from build123d import *

# Parameters (mm, degrees)
WEB_RECESS_SKETCH_R       = 100
WEB_RECESS_200_DEPTH      = 28
LIGHTENING_HOLES_SKETCH_R = 18
LIGHTENING_HOLES_4X_DEPTH = 11
HUB_SKETCH_R              = 25
HUB_50_DEPTH              = 35
BORE_SKETCH_R             = 12.5
BORE_25_DEPTH             = 35
KEYWAY_SKETCH_W           = 3
KEYWAY_SKETCH_H           = 6
KEYWAY_6X3_DEPTH          = 35


with BuildPart() as part:
    # Pulley Profile Sketch → Pulley Body 3-Groove (revolve)
    with BuildSketch(Plane.XY, mode=Mode.PRIVATE) as pulley_body_3_groove_sk:
        Polygon((-38.155633051, 12.5), (38.155633051, 12.5), (38.155633051, 125), (33.155633051, 125), (26.604168834, 107), (20.629224678, 107.05281598), (14.096983906, 125), (9.096983906, 125), (2.5, 106.874935681), (-2.5, 106.874935681), (-9.096983906, 125), (-14.096983906, 125), (-20.629224678, 107.05281598), (-26.604168834, 107), (-33.155633051, 125), (-38.155633051, 125), align=None)
    revolve(pulley_body_3_groove_sk.sketch.rotate(Axis((-177.514342584, 0, 0), (1, 0, 0)), 90), axis=Axis((-177.514342584, 0, 0), (1, 0, 0)))

    # Web Recess Sketch → Web Recess Ø200 (cut)
    with BuildSketch(Plane(origin=(38.155633051, 0, 0), x_dir=(0, 0, -1), z_dir=(1, 0, 0))):
        Circle(WEB_RECESS_SKETCH_R)
    web_recess_200 = extrude(amount=-WEB_RECESS_200_DEPTH, mode=Mode.SUBTRACT)

    # Web Recess Mirror: Web Recess Ø200 across plane
    add(web_recess_200.mirror(Plane(origin=(0, 0, 0), x_dir=(0, 0, 1), z_dir=(1, 0, 0))), mode=Mode.SUBTRACT)

    # Lightening Holes Sketch → Lightening Holes 4x (cut, symmetric)
    with BuildSketch(Plane(origin=(0, 0, 0), x_dir=(0, 0, -1), z_dir=(1, 0, 0))):
        with Locations((0, 62.5)):
            Circle(LIGHTENING_HOLES_SKETCH_R)
        with Locations((62.5, 0)):
            Circle(LIGHTENING_HOLES_SKETCH_R)
        with Locations((0, -62.5)):
            Circle(LIGHTENING_HOLES_SKETCH_R)
        with Locations((-62.5, 0)):
            Circle(LIGHTENING_HOLES_SKETCH_R)
    extrude(amount=LIGHTENING_HOLES_4X_DEPTH, both=True, mode=Mode.SUBTRACT)

    # Hub Sketch → Hub Ø50 (add, symmetric)
    with BuildSketch(Plane(origin=(0, 0, 0), x_dir=(0, 0, -1), z_dir=(1, 0, 0))):
        with Locations(Location((0, 0, 0), (0, 0, 180))):
            Circle(HUB_SKETCH_R)
    extrude(amount=HUB_50_DEPTH, both=True)

    # Bore Sketch → Bore Ø25 (cut, symmetric)
    with BuildSketch(Plane(origin=(0, 0, 0), x_dir=(0, 0, -1), z_dir=(1, 0, 0))):
        Circle(BORE_SKETCH_R)
    extrude(amount=BORE_25_DEPTH, both=True, mode=Mode.SUBTRACT)

    # Keyway Sketch → Keyway 6x3 (cut, symmetric)
    with BuildSketch(Plane(origin=(0, 0, 0), x_dir=(0, 0, -1), z_dir=(1, 0, 0))):
        with Locations((13.6346611, 0)):
            Rectangle(KEYWAY_SKETCH_W, KEYWAY_SKETCH_H)
    extrude(amount=KEYWAY_6X3_DEPTH, both=True, mode=Mode.SUBTRACT)


solid = part.part
Read the model definition and answer for the solid it produces. Units are mm, in the model's axes. A direction names the side the tool comes from. Round coordinates to 2 decimals unless told otherwise and drop trailing zeros.
Q1. Each of these flat-tipped pins is pushed along its axis until it touches: pin 1 (2.5 mm diameter, centred on x = -12, z = -13, fed in from +Y); pin 2 (25 mm diameter, centred on y = 10, z = -0.5, fed in from -X); pin 3 (10 mm diameter, centred on x = 14.5, y = 82.5, fed in from +Z); pin 4 (21.5 mm diameter, centred on y = 62.5, z = 0, fed in from -X). Where does it stop, or does it pass through?
Q2. Which of the six approach directions +Z, -Z, +X, -X, +Y, -Y give full straight-line access (tool end or side, diameter ignored) to faces 5 (the face through (0.142, -44.653, 2.343)), 6 (the face through (24.239, -32.146, 102.079)), 7 (the face through (35, -11.5, -5.9)), 8 (the face through (-35, -11.5, -5.9))?
Q3. Section A-A on y = 0 is taken. Give the number of separate pieces and of enclosed holes in the cut face, and give its area (3 significant figures).
Q4. Consider probe 1 along Y at (x, z) = (-2, 0); probe 2 along X at (y, z) = (-96.5, -79); probe 3 along X at (y, z) = (68, 91). Determine where each line is inside the solid, lowest interval first.
Q5. Determine the mould class of faces 1 (the face through (-22.404, -7.509, 23.846)), 2 (the face through (2.82, 65.57, -85.51)), 3 (the face through (-10.156, -21, -21)), 4 (the face through (38.156, -84, 56)) for opening direction X: released by +X, released by -X, zero draft, split by the parting line, or undercut.
Output:
1. pin 1: stops at y = 124.45
1. pin 2: stops at x = -35
1. pin 3: stops at z = 98.06
1. pin 4: passes through
2. face 5: +X, -X
2. face 6: none
2. face 7: +X
2. face 8: -X
3. separate pieces: 4
3. enclosed holes: 0
3. area: 5,650 mm2
4. probe 1: y = -106.87 to -80.5, -44.5 to -12.5, 12.5 to 44.5, 80.5 to 106.87
4. probe 2: x = -38.16 to -33.05, -14.2 to -8.99, 8.99 to 14.2, 33.05 to 38.16
4. probe 3: x = -38.16 to -29.01, -18.25 to -4.95, 4.95 to 18.25, 29.01 to 38.16
5. face 1: zero draft
5. face 2: undercut
5. face 3: released by -X
5. face 4: released by +X
